Geometry: final body of the model. Coordinates: model frame, mm. Face numbers are marked on the shaded views. Give positions to 0.01 mm unless a question says otherwise; leave off trailing zeros. Loops run counter-clockwise (first coordinate to the right, second up) from the corner with the lowest first, then second, coordinate; pieces in that order, holes last.
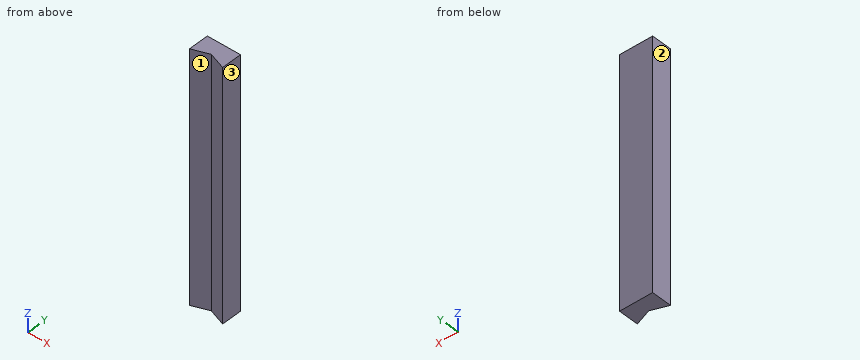
from build123d import *

# Parameters (mm, degrees)
EXTRUDE_1_DEPTH = 105


with BuildPart() as part:
    # 草图1 → 凸台-拉伸1 (new, symmetric)
    with BuildSketch(Plane.XY):
        Polygon((0, 0), (-14, -5), (-14, 12), (14, 12), (14, -5), align=None)
    extrude(amount=EXTRUDE_1_DEPTH, both=True)


solid = part.part
Item 1: Section query A-A on z = 18.5. Return loops of the section in (x, y), plus the area to 3 significant figures.
Values follow:
outline: (-14, -5) - (0, 0) - (14, -5) - (14, 12) - (-14, 12) - close
area: 406 mm2
Item 2: Section query C-C on x = -7. Return loops of the section in (y, z).
Values follow:
outline: (-2.5, -105) - (12, -105) - (12, 105) - (-2.5, 105) - close
Item 3: Draft query along X for the marked faces 1, 2 and 3. Return one class per face: +X half, -X half, draft (parallel to the pull), parting line (faces both ways), or undercut.
Values follow:
face 1: undercut
face 2: -X half
face 3: +X half
Item 4: Ray query, probe 1 along Y at (x, z) = (-12.25, 14) (3 decimals); probe 2 along Y at (x, z) = (-0.5, 71). Return the intervals inside material, ascending.
Values follow:
probe 1: y = -4.375 to 12
probe 2: y = -0.18 to 12
Item 5: Pin query (flat end, axial travel): pin 1 (1 mm diameter, centred on x = 8, z = -58.5, fed in from -Y); pin 2 (3 mm diameter, centred on x = -0.5, z = 69, fed in from -Y). Return the tip coordinate at first contact, or that it passes through.
Values follow:
pin 1: stops at y = -3.04
pin 2: stops at y = -0.71
Item 6: Section query B-B on x = 10.5. Return loops of the section in (y, z), plus the area to 3 significant figures.
Values follow:
outline: (-3.75, -105) - (12, -105) - (12, 105) - (-3.75, 105) - close
area: 3,310 mm2
